CAD build for the part. Positions are in the model's coordinates, mm. Coordinates: 2 decimals unless noted, no trailing zeros. Order: outer loops, then holes, each group sorted by start corner. A loop starts at its lowest first (then second) coordinate and runs counter-clockwise, first axis right, second up. Notation, with made-up numbers: M -32.75,64.5 L 19.25,64.5 A12 ccw 19.25,77.5 Z; hole C -27.75,-5 d2. An arc over 180 degrees is marked long. Write item = value, one per line. Start each with the question number.
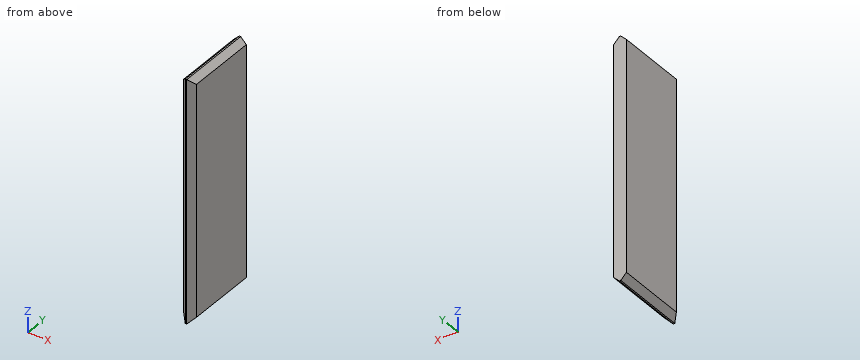
```python
from build123d import *

# Parameters (mm, degrees)
SKETCH1_W           = 850
SKETCH1_H           = 265
BOSS_EXTRUDE1_DEPTH = 22.5
CHAMFER1_SIZE       = 20


with BuildPart() as part:
    # Sketch1 → Boss-Extrude1 (new, symmetric)
    with BuildSketch(Plane(origin=(0, 0, 0), x_dir=(0, 0, -1), z_dir=(1, 0, 0))):
        Rectangle(SKETCH1_W, SKETCH1_H)
    extrude(amount=BOSS_EXTRUDE1_DEPTH, both=True)

    # Chamfer1
    chamfer1_edges = [part.edges().sort_by_distance(p)[0] for p in [
        (22.5, 0, -425),
        (22.5, 0, 425),
        (-22.5, 0, -425),
        (-22.5, -132.5, 0),
        (-22.5, 0, 425),
        (22.5, -132.5, 0),
    ]]
    chamfer(chamfer1_edges, length=CHAMFER1_SIZE)


solid = part.part
```
1. Slice it at B-B (z = -89). Write the cut outline in (x, y), plus the area to 3 significant figures.
2. Probe L1, parallel to Z at x = 9, y = -39; L2, parallel to Y at x = -17, z = -269; L3, parallel to Z at x = 16.5, y = 107.5. List the from-to ranges inside material, lowest first.
3. Slice it at C-C (x = 11.5). Write the cut outline in (y, z).
4. Flat gauge pins, fed straight in: pin 1 (4 mm diameter, centred on x = 10.5, z = -174.5, fed in from -Y); pin 2 (4 mm diameter, centred on x = 17.5, z = 195, fed in from -Y); pin 3 (5 mm diameter, centred on x = -12, y = 45.5, fed in from +Z). Where does each tip first touch, or does it go through?
5. Slice it at A-A (y = 15). Write the cut outline in (x, z), plus the area to 4 significant figures.
Calculated:
q1.outline = M -22.5,-112.5 L -2.5,-132.5 L 2.5,-132.5 L 22.5,-112.5 L 22.5,132.5 L -22.5,132.5 Z
q1.area = 11,500 mm²
q2.L1 = -418.5 to 418.5
q2.L2 = -118 to 132.5
q2.L3 = -411 to 411
q3.outline = M -123.5,-416 L 132.5,-416 L 132.5,416 L -123.5,416 Z
q4.pin_1 = -126.5
q4.pin_2 = -119.5
q4.pin_3 = 418
q5.outline = M -22.5,-405 L -2.5,-425 L 2.5,-425 L 22.5,-405 L 22.5,405 L 2.5,425 L -2.5,425 L -22.5,405 Z
q5.area = 37,450 mm²
